```python
from build123d import *

# Parameters (mm, degrees)
BOSS_EXTRUDE1_DEPTH   = 2.5
M5_TAPPED_HOLE1_D     = 4.2
M5_TAPPED_HOLE1_DEPTH = 5
M5_TAPPED_HOLE1_TIP   = 1.2618073


with BuildPart() as part:
    # Sketch1 → Boss-Extrude1 (new, symmetric)
    with BuildSketch(Plane(origin=(0, 0, 0), x_dir=(0, 0, -1), z_dir=(1, 0, 0))):
        with BuildLine():
            Line((-15, 210), (-39.5, 210))
            ThreePointArc((-39.5, 210), (-49.5, 200), (-39.5, 190))
            Line((-39.5, 190), (-15, 190))
            Line((-15, 190), (-15, 210))
        make_face()
    extrude(amount=BOSS_EXTRUDE1_DEPTH, both=True)

    # M5 Tapped Hole1
    with Locations(Plane(origin=(-2.5, 200, 39.5), x_dir=(0, 0, -1), z_dir=(-1, 0, 0))):
        with Locations((0, 0)):
            Hole(M5_TAPPED_HOLE1_D / 2, depth=M5_TAPPED_HOLE1_DEPTH)
            with Locations((0, 0, -(M5_TAPPED_HOLE1_DEPTH + M5_TAPPED_HOLE1_TIP / 2))):  # 118° drill point
                Cone(0, M5_TAPPED_HOLE1_D / 2, M5_TAPPED_HOLE1_TIP, mode=Mode.SUBTRACT)


solid = part.part
```
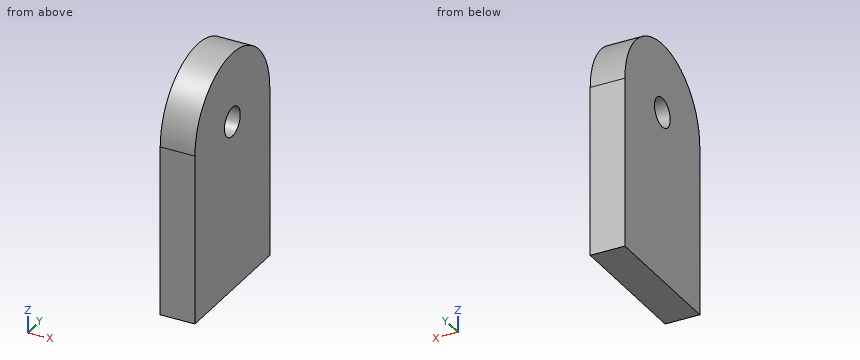
The model under review builds one solid part; all positions refer to its coordinate system, in mm. Round coordinates to 2 decimals unless told otherwise and drop trailing zeros. Write each loop counter-clockwise with the first axis right and the second up, starting at its lowest first coordinate (ties: lowest second). Pieces come first, ordered by that corner, then holes.
(1) Wall thickness on L1, parallel to Y at x = -1.05, z = 39.5; L2, parallel to Z at x = -0.7, y = 200; L3, parallel to Z at x = 1.75, y = 201.5: over which ranges is each line inside the solid? List them lowest first.
(2) We need section C-C on z = 40.5. Give the boundary of the cut face in (x, y), and give its area (3 significant figures).
(3) We need section A-A on y = 200. Give the boundary of the cut face in (x, z).
(4) We need section D-D on y = 195.75. Give the boundary of the cut face in (x, z).
(5) We need section B-B on x = -1.25. Give the boundary of the cut face in (y, z), and give its area (3 significant figures).
Findings below:
1. L1: y = 190 to 197.9, 202.1 to 210
1. L2: z = 15 to 37.4, 41.6 to 49.5
1. L3: z = 15 to 38.03, 40.97 to 49.39
2. outline: (-2.5, 190.05) - (2.5, 190.05) - (2.5, 198.15) - (-2.5, 198.15) - close; (-2.5, 201.85) - (2.5, 201.85) - (2.5, 209.95) - (-2.5, 209.95) - close
2. area: 81.0 mm2
3. outline: (-2.5, 15) - (2.5, 15) - (2.5, 37.4) - (-2.5, 37.4) - close; (-2.5, 41.6) - (2.5, 41.6) - (2.5, 49.5) - (-2.5, 49.5) - close
4. outline: (-2.5, 15) - (2.5, 15) - (2.5, 48.55) - (-2.5, 48.55) - close
5. outline: (190, 15) - (210, 15) - (210, 39.5) arc R10 ccw to (190, 39.5) - close; hole circle Ø4.2 at (200, 39.5)
5. area: 633 mm2
